Build history of the part. All positions in model axes, mm. Face numbers are marked on the shaded views. A direction names the side the tool comes from. Round coordinates to 2 decimals unless told otherwise and drop trailing zeros. Write each loop counter-clockwise with the first axis right and the second up, starting at its lowest first coordinate (ties: lowest second). Pieces come first, ordered by that corner, then holes. Notation, with made-up numbers: M -9,-25 L 27,-25 A15 cw 27,-1 Z; hole C 39.5,-11 d7. An arc over 180 degrees is marked long. Write item = value, one per line. Start each with the question number.
Q1. Band-saw the part on A-A on z = 0. Write the cut outline in (x, y), plus the area to 3 significant figures.
Q2. Band-saw the part on D-D on y = 93.5. Write the cut outline in (x, z), plus the area to 3 significant figures.
Q3. Band-saw the part on B-B on x = 0. Write the cut outline in (y, z), plus the area to 3 significant figures.
Q4. Tool access for the marked faces 1, 2 and 3: list every direction of +Z, -Z, +X, -X, +Y, -Y with a clear straight run to the whole face (end or side of a thin tool).
Q5. Drop flat-ended pins along their axis: P1, Ø4, axis at x = 26, y = 7, coming from the +Z side; P2, Ø2, axis at y = 51.5, z = -29.5, coming from the -X side; P3, Ø1.5, axis at y = 59.5, z = 0, coming from the -X side. Give the stop position or say it passes through.
Q6. Probe L1, parallel to Z at x = 9.5, y = -40.5; L2, parallel to X at y = -46, z = -0.5; L3, parallel to X at y = -82, z = -2. List the from-to ranges inside material, lowest first.
Q7. Band-saw the part on C-C on y = -4.5. Write the cut outline in (x, z), plus the area to 3 significant figures.
```python
from build123d import *

# Parameters (mm, degrees)
SKETCH1_R           = 50
BOSS_EXTRUDE1_DEPTH = 120
SKETCH2_R           = 50
SKETCH2_R_2         = 40
CUT_EXTRUDE1_DEPTH  = 36
CUT_EXTRUDE2_START  = -37
SKETCH3_R           = 50
SKETCH3_R_2         = 40
CUT_EXTRUDE2_DEPTH  = 37
SKETCH4_R           = 50
SKETCH4_R_2         = 45
CUT_EXTRUDE3_DEPTH  = 134
CHAMFER1_SIZE       = 3
CHAMFER2_SIZE       = 1


with BuildPart() as part:
    # Sketch1 → Boss-Extrude1 (new, symmetric)
    with BuildSketch(Plane(origin=(0, 0, 0), x_dir=(1, 0, 0), z_dir=(0, 1, 0))):
        with Locations(Location((0, 0, 0), (0, 0, 270))):
            Circle(SKETCH1_R)
    extrude(amount=BOSS_EXTRUDE1_DEPTH, both=True)

    # Sketch2 → Cut-Extrude1 (cut)
    with BuildSketch(Plane(origin=(0, 120, 0), x_dir=(1, 0, 0), z_dir=(0, 1, 0))):
        with Locations(Location((0, 0, 0), (0, 0, 270))):
            Circle(SKETCH2_R)
        with Locations(Location((0, 0, 0), (0, 0, 270))):
            Circle(SKETCH2_R_2, mode=Mode.SUBTRACT)
    extrude(amount=-CUT_EXTRUDE1_DEPTH, mode=Mode.SUBTRACT)

    # Sketch3 → Cut-Extrude2 (cut)
    with BuildSketch(Plane.XZ.offset(120).offset(CUT_EXTRUDE2_START)):
        with Locations(Location((0, 0, 0), (0, 0, 270))):
            Circle(SKETCH3_R)
        with Locations(Location((0, 0, 0), (0, 0, 90))):
            Circle(SKETCH3_R_2, mode=Mode.SUBTRACT)
    extrude(amount=CUT_EXTRUDE2_DEPTH, mode=Mode.SUBTRACT)

    # Sketch4 → Cut-Extrude3 (cut)
    with BuildSketch(Plane(origin=(0, 84, 0), x_dir=(1, 0, 0), z_dir=(0, 1, 0))):
        with Locations(Location((0, 0, 0), (0, 0, 90))):
            Circle(SKETCH4_R)
        with Locations(Location((0, 0, 0), (0, 0, 270))):
            Circle(SKETCH4_R_2, mode=Mode.SUBTRACT)
    extrude(amount=-CUT_EXTRUDE3_DEPTH, mode=Mode.SUBTRACT)

    # Chamfer1
    chamfer1_edges = [part.edges().sort_by_distance(p)[0] for p in [
        (0, -120, -40),
        (0, 120, -40),
    ]]
    chamfer(chamfer1_edges, length=CHAMFER1_SIZE)

    # Chamfer2
    chamfer2_edges = [part.edges().sort_by_distance(p)[0] for p in [
        (0, -83, -50),
        (0, -50, -50),
        (0, 84, -45),
    ]]
    chamfer(chamfer2_edges, length=CHAMFER2_SIZE)


solid = part.part
```
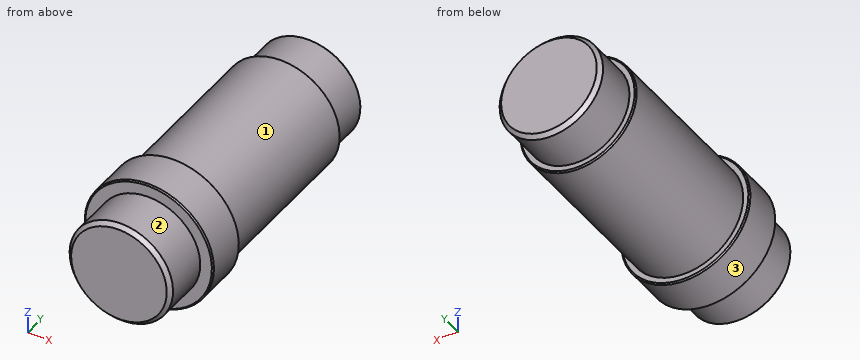
Conclusion:
q1.outline = M -50,-82 L -49,-83 L -40,-83 L -40,-117 L -37,-120 L 37,-120 L 40,-117 L 40,-83 L 49,-83 L 50,-82 L 50,-51 L 49,-50 L 45,-50 L 45,83 L 44,84 L 40,84 L 40,117 L 37,120 L -37,120 L -40,117 L -40,84 L -44,84 L -45,83 L -45,-50 L -49,-50 L -50,-51 Z
q1.area = 21,200 mm^2
q2.outline = C 0,0 d80
q2.area = 5,030 mm^2
q3.outline = M -120,-37 L -117,-40 L -83,-40 L -83,-49 L -82,-50 L -51,-50 L -50,-49 L -50,-45 L 83,-45 L 84,-44 L 84,-40 L 117,-40 L 120,-37 L 120,37 L 117,40 L 84,40 L 84,44 L 83,45 L -50,45 L -50,49 L -51,50 L -82,50 L -83,49 L -83,40 L -117,40 L -120,37 Z
q3.area = 21,200 mm^2
q4.face_1 = +Y
q4.face_2 = -Y
q4.face_3 = +Y, -Y
q5.P1 = 38.07
q5.P2 = -34.82
q5.P3 = -45
q6.L1 = -43.99 to 43.99
q6.L2 = -45 to 45
q6.L3 = -49.96 to 49.96
q7.outline = C 0,0 d90
q7.area = 6,360 mm^2
